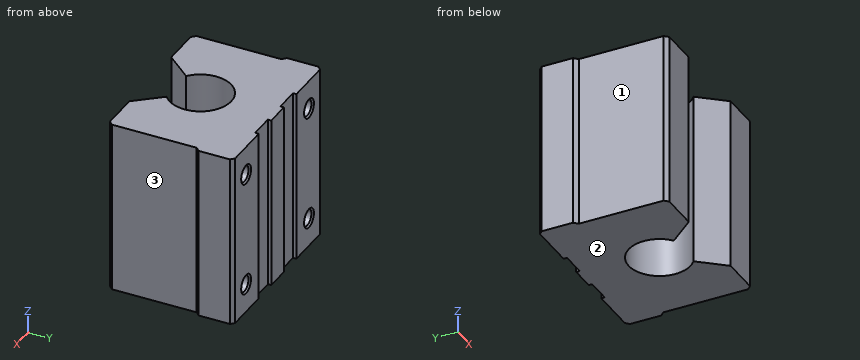
```python
from build123d import *

# Parameters (mm, degrees)
SKETCH_1_W               = 45
SKETCH_1_H               = 45
EXTRUDE_1_DEPTH          = 33
SKETCH_2_W               = 6.4
SKETCH_2_H               = 0.9
CUT_EXTRUDE_1_DEPTH      = 68.5
SKETCH_3_W               = 6.4
SKETCH_3_H               = 0.9
CUT_EXTRUDE_2_DEPTH      = 68.5
SKETCH_4_W               = 1
SKETCH_4_H               = 24
CUT_EXTRUDE_3_DEPTH      = 68.5
CUT_EXTRUDE_4_DEPTH      = 68.5
SKETCH_6_W               = 1
SKETCH_6_H               = 24
CUT_EXTRUDE_5_DEPTH      = 68.500000167
DRAFT_1_ANGLE            = 45
DRAFT_2_ANGLE            = 45
DRAFT_3_ANGLE            = 40
HOLE_WIZARD_16_0_16_1_D  = 16.000000007
HOLE_WIZARD_M3_5_1_D     = 4.134
HOLE_WIZARD_M3_5_1_DEPTH = 15.60662
HOLE_WIZARD_M3_5_1_TIP   = 1.193383006
CHAMFER_1_SIZE           = 0.433
CHAMFER_2_SIZE           = 1
CHAMFER_3_SIZE           = 0.9
CUT_EXTRUDE_6_DEPTH      = 106.297198595


with BuildPart() as part:
    # 草图1 → 凸台-拉伸1 (new body)
    with BuildSketch(Plane.XZ.offset(-12)):
        with Locations((0, 230)):
            Rectangle(SKETCH_1_W, SKETCH_1_H)
    extrude(amount=-EXTRUDE_1_DEPTH)

    # 草图2 → 切除-拉伸1 (cut, through all)
    with BuildSketch(Plane.XY.offset(252.5)):
        with Locations((-6.4, 44.55)):
            Rectangle(SKETCH_2_W, SKETCH_2_H)
    extrude(amount=-CUT_EXTRUDE_1_DEPTH, mode=Mode.SUBTRACT)

    # 草图3 → 切除-拉伸2 (cut, through all)
    with BuildSketch(Plane.XY.offset(252.5)):
        with Locations((6.4, 44.55)):
            Rectangle(SKETCH_3_W, SKETCH_3_H)
    extrude(amount=-CUT_EXTRUDE_2_DEPTH, mode=Mode.SUBTRACT)

    # 草图4 → 切除-拉伸3 (cut, through all)
    with BuildSketch(Plane.XY.offset(252.5)):
        with Locations((22, 24)):
            Rectangle(SKETCH_4_W, SKETCH_4_H)
    extrude(amount=-CUT_EXTRUDE_3_DEPTH, mode=Mode.SUBTRACT)

    # 草图5 → 切除-拉伸4 (cut, through all)
    with BuildSketch(Plane.XY.offset(252.5)):
        with BuildLine():
            Line((-10.668119688, 12), (10.668119688, 12))
            add(Edge.make_bspline(
                [(5, 18.755002002), (6.889373229, 16.503334668), (8.778746459, 14.251667334), (10.668119688, 12)],
                knots=[0, 0, 0, 0, 1, 1, 1, 1], degree=3))
            Line((5, 18.755002002), (-10.668119688, 37.427539929))
            Line((-10.668119688, 37.427539929), (-10.668119688, 12))
        make_face()
    extrude(amount=-CUT_EXTRUDE_4_DEPTH, mode=Mode.SUBTRACT)

    # 草图6 → 切除-拉伸5 (cut, through all)
    with BuildSketch(Plane.XY.offset(252.5)):
        with Locations((-22, 24)):
            Rectangle(SKETCH_6_W, SKETCH_6_H)
    extrude(amount=-CUT_EXTRUDE_5_DEPTH, mode=Mode.SUBTRACT)

    # 拔模1
    draft_1_faces = [part.faces().sort_by_distance(p)[0] for p in [
        (-22, 36, 230),
    ]]
    draft(draft_1_faces, Plane(origin=(-22.5, 45, 252.5), x_dir=(0, 0, -1), z_dir=(-1, 0, 0)), DRAFT_1_ANGLE)

    # 拔模2
    draft_2_faces = [part.faces().sort_by_distance(p)[0] for p in [
        (22, 36, 230),
    ]]
    draft(draft_2_faces, Plane(origin=(22.5, 45, 207.5), x_dir=(0, 0, 1), z_dir=(1, 0, 0)), DRAFT_2_ANGLE)

    # 拔模3
    draft_3_faces = [part.faces().sort_by_distance(p)[0] for p in [
        (-10.668119688, 24.713769965, 230),
    ]]
    draft(draft_3_faces, Plane(origin=(0, 12, 0), x_dir=(0, 0, -1), z_dir=(0, -1, 0)), DRAFT_3_ANGLE)

    # Ø16.0 (16) 直径孔1 (through all)
    with Locations(Plane(origin=(0, 0, 207.5), x_dir=(-1, 0, 0), z_dir=(0, 0, -1))):
        with Locations((0, 25)):
            Hole(HOLE_WIZARD_16_0_16_1_D / 2)

    # M3.5 间隙孔1
    with Locations(Plane(origin=(0, 45, 0), x_dir=(1, 0, 0), z_dir=(0, 1, 0))):
        with Locations((16, -215), (16, -245), (-16, -215), (-16, -245)):
            Hole(HOLE_WIZARD_M3_5_1_D / 2, depth=HOLE_WIZARD_M3_5_1_DEPTH)
            with Locations((0, 0, -(HOLE_WIZARD_M3_5_1_DEPTH + HOLE_WIZARD_M3_5_1_TIP / 2))):  # 120° drill point
                Cone(0, HOLE_WIZARD_M3_5_1_D / 2, HOLE_WIZARD_M3_5_1_TIP, mode=Mode.SUBTRACT)

    # 倒角1
    chamfer_1_edges = [part.edges().sort_by_distance(p)[0] for p in [
        (-13.933, 45, 245),
        (-13.933, 45, 215),
        (18.067, 45, 245),
        (18.067, 45, 215),
    ]]
    chamfer(chamfer_1_edges, length=CHAMFER_1_SIZE)

    # 倒角2
    chamfer_2_edges = [part.edges().sort_by_distance(p)[0] for p in [
        (21.5, 12, 230),
        (-21.5, 12, 230),
    ]]
    chamfer(chamfer_2_edges, length=CHAMFER_2_SIZE)

    # 倒角3
    chamfer_3_edges = [part.edges().sort_by_distance(p)[0] for p in [
        (-22.5, 45, 230),
        (22.5, 45, 230),
    ]]
    chamfer(chamfer_3_edges, length=CHAMFER_3_SIZE)

    # 草图11 → 切除-拉伸6 (cut, through all)
    with BuildSketch(Plane.XY.offset(300)):
        with BuildLine():
            Line((-9.25, 11.7), (-9.25, 5))
            Line((-9.25, 5), (-20, 5))
            Line((-20, 5), (-20, 0))
            Line((-20, 0), (20, 0))
            Line((20, 0), (20, 5))
            Line((20, 5), (9.25, 5))
            Line((9.25, 5), (9.25, 11.7))
            Line((9.25, 11.7), (9.11850775, 11.7))
            Line((9.11850775, 11.7), (4, 17.8))
            Line((4, 17.8), (3.487119155, 17.8))
            ThreePointArc((3.487119155, 17.8), (0, 33), (-3.487119155, 17.8))
            Line((-3.487119155, 17.8), (-4, 17.8))
            Line((-4, 17.8), (-9.11850775, 11.7))
            Line((-9.11850775, 11.7), (-9.25, 11.7))
        make_face()
    extrude(amount=-CUT_EXTRUDE_6_DEPTH, mode=Mode.SUBTRACT)


solid = part.part
```
Input: part model. Units: mm. Frame: model coordinates. Face numbers are marked on the shaded views. A direction names the side the tool comes from. Round coordinates to 2 decimals unless told otherwise and drop trailing zeros. Loops run counter-clockwise (first coordinate to the right, second up) from the corner with the lowest first, then second, coordinate; pieces in that order, holes last.
1) Section query A-A on y = 25. Return the cut outline in (x, z).
Ans:
outline: (-21.5, 207.5) - (-8, 207.5) - (-8, 252.5) - (-21.5, 252.5) - close; (8, 207.5) - (21.5, 207.5) - (21.5, 252.5) - (8, 252.5) - close
2) Set-up query: the marked faces 1, 2 and 3. Return all of +Z, -Z, +X, -X, +Y, -Y with unobstructed straight access to the full face (end or side cutting, diameter ignored); none if empty.
Ans:
face 1: +Z, -Z, -X, -Y
face 2: -Z, +X, -X, +Y, -Y
face 3: +Z, -Z, +X, -Y
3) Pin query (flat end, axial travel): pin 1 (0.7 mm diameter, centred on y = 45, z = 240, fed in from +X); pin 2 (1 mm diameter, centred on y = 21, z = 245, fed in from -X); pin 3 (0.7 mm diameter, centred on y = 44.5, z = 220.5, fed in from -X). Return the tip coordinate at first contact, or that it passes through.
Ans:
pin 1: stops at x = 21.95
pin 2: stops at x = -21.5
pin 3: stops at x = -22.45
4) Section query D-D on x = 1. Return the cut outline in (y, z), plus the area to 3 significant figures.
Ans:
outline: (32.94, 207.5) - (45, 207.5) - (45, 252.5) - (32.94, 252.5) - close
area: 543 mm2
5) Section query C-C on x = -4. Return the cut outline in (y, z).
Ans:
outline: (31.93, 207.5) - (44.1, 207.5) - (44.1, 252.5) - (31.93, 252.5) - close
6) Material intervals for line 1 (Z direction, x = 16, y = 37.5); line 2 (X direction, y = 41.75, z = 215); line 3 (X direction, y = 25, z = 242.5), sorted ascending.
Ans:
line 1: z = 207.5 to 212.93, 217.07 to 242.93, 247.07 to 252.5
line 2: x = -22.5 to -18.07, -13.93 to 13.93, 18.07 to 22.5
line 3: x = -21.5 to -8, 8 to 21.5
7) Section query B-B on y = 21. Return the cut outline in (x, z), plus the area to 3 significant figures.
Ans:
outline: (-21.5, 207.5) - (-6.93, 207.5) - (-6.93, 252.5) - (-21.5, 252.5) - close; (6.93, 207.5) - (21.5, 207.5) - (21.5, 252.5) - (6.93, 252.5) - close
area: 1,310 mm2
